Could you check a few things on this model? Use its own coordinates, in mm. Face numbers are marked on the shaded views. Give positions to 0.01 mm unless a question says otherwise; leave off trailing zeros. Order: outer loops, then holes, each group sorted by start corner. A loop starts at its lowest first (then second) coordinate and runs counter-clockwise, first axis right, second up. Notation, with made-up numbers: M -22,85 L -18,85 A9 cw -18,93 Z; hole C 87.25,60.25 d7. An arc over 180 degrees is marked long. Use a Markdown table: item, result. Add a question column.
Item 1: If I drill on L1, parallel to Z at x = -17.5, y = 7; L2, parallel to Y at x = 0, z = 5; L3, parallel to Z at x = -17.5, y = -8.25, over which ranges is the centre line in solid material (lowest first)? Write a range as from..to.
Item 2: Suppose I cut it at B-B on x = -17.5. Write out the boundary of the cut face in (y, z), plus the area to 3 significant figures.
Item 3: Suppose I cut it at D-D on y = 7. Write out the boundary of the cut face in (x, z).
Item 4: Suppose I cut it at C-C on y = 0. Write out the boundary of the cut face in (x, z).
Item 5: If we mould it in two halves opening along Z, with no side actions, what happens to the marked faces 1, 2, 3 and 4? For each: released by +Z, released by -Z, zero draft, split by the parting line, or undercut.
Item 6: I'm going to push a flat-ended pin straight in: pin 1 Ø7 at (x, z) = (-17.5, 7.5) entering from -Y. Where does the tip first touch, or does it pass through?
Item 7: Suppose I cut it at A-A on z = 7.5. Write out the boundary of the cut face in (x, y), plus the area to 3 significant figures.
from build123d import *

# Parameters (mm, degrees)
SKETCH_1_W                   = 50
SKETCH_1_H                   = 25
EXTRUDE_1_DEPTH              = 15
CHAMFER_1_SIZE               = 2
HOLE_WIZARD_M5_1_D           = 5.5
HOLE_WIZARD_M5_1_CBORE_D     = 10
HOLE_WIZARD_M5_1_CBORE_DEPTH = 15.7
HOLE_WIZARD_M8_1_D           = 6.8


with BuildPart() as part:
    # 草图1 → 凸台-拉伸1 (new body)
    with BuildSketch(Plane.XY):
        Rectangle(SKETCH_1_W, SKETCH_1_H)
    extrude(amount=EXTRUDE_1_DEPTH)

    # 倒角1
    chamfer_1_edges = [part.edges().sort_by_distance(p)[0] for p in [
        (25, -12.5, 7.5),
        (-25, -12.5, 7.5),
    ]]
    chamfer(chamfer_1_edges, length=CHAMFER_1_SIZE)

    # M5 六角圆柱头螺钉的柱形沉头孔1 (through all)
    with Locations(Plane(origin=(0, -12.5, 0), x_dir=(-1, 0, 0), z_dir=(0, -1, 0))):
        with Locations((-17.5, -7.5), (17.5, -7.5)):
            CounterBoreHole(HOLE_WIZARD_M5_1_D / 2, HOLE_WIZARD_M5_1_CBORE_D / 2, HOLE_WIZARD_M5_1_CBORE_DEPTH)

    # M8 螺纹孔1 (through all)
    with Locations(Plane.XY.offset(15)):
        with Locations((0, 0)):
            Hole(HOLE_WIZARD_M8_1_D / 2)


solid = part.part
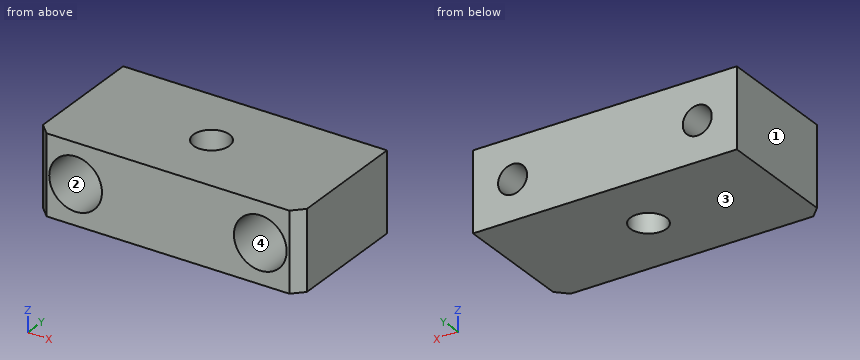
Findings below:
| question | item | result |
|---|---|---|
| 1 | L1 | z = 0..4.75, 10.25..15 |
| 1 | L2 | y = -12.5..-3.4, 3.4..12.5 |
| 1 | L3 | z = 0..2.5, 12.5..15 |
| 2 | outline | M -12.5,0 L 12.5,0 L 12.5,4.75 L 3.2,4.75 L 3.2,2.5 L -12.5,2.5 Z; M -12.5,12.5 L 3.2,12.5 L 3.2,10.25 L 12.5,10.25 L 12.5,15 L -12.5,15 Z |
| 2 | area | 167 mm^2 |
| 3 | outline | M -25,0 L 25,0 L 25,15 L -25,15 Z; hole C -17.5,7.5 d5.5; hole C 17.5,7.5 d5.5 |
| 4 | outline | M -25,0 L -3.4,0 L -3.4,15 L -25,15 Z; M 3.4,0 L 25,0 L 25,15 L 3.4,15 Z; hole C -17.5,7.5 d10; hole C 17.5,7.5 d10 |
| 5 | face 1 | zero draft |
| 5 | face 2 | undercut |
| 5 | face 3 | released by -Z |
| 5 | face 4 | undercut |
| 6 | pin 1 | stops at y = 3.2 |
| 7 | outline | M -25,-10.5 L -23,-12.5 L -22.5,-12.5 L -22.5,3.2 L -20.25,3.2 L -20.25,12.5 L -25,12.5 Z; M -14.75,3.2 L -12.5,3.2 L -12.5,-12.5 L 12.5,-12.5 L 12.5,3.2 L 14.75,3.2 L 14.75,12.5 L -14.75,12.5 Z; M 20.25,3.2 L 22.5,3.2 L 22.5,-12.5 L 23,-12.5 L 25,-10.5 L 25,12.5 L 20.25,12.5 Z; hole C 0,0 d6.8 |
| 7 | area | 793 mm^2 |
